Job drawing, mm, ordinate dimensions from the low corner. One solid piece. Give positions to 0.01 mm unless a question says otherwise; leave off trailing zeros. Loops run counter-clockwise (first coordinate to the right, second up) from the corner with the lowest first, then second, coordinate; pieces in that order, holes last.
Item 1: Saw through at B-B on x = 245. Give the cut face in (y, z).
Item 2: Probe probe 1 along Y at (x, z) = (245, 15); probe 2 along Y at (x, z) = (48, 21). List the from-to ranges inside material, lowest first.
Item 3: Drop a flat-ended pin along its axis: P1, Ø16, axis at x = 245, y = 110, coming from the +Z side. Give the stop position or say it passes through.
Item 4: Saw through at C-C on y = 30. Give the cut face in (x, z), plus the area to 3 significant figures.
Item 5: Saw through at A-A on z = 24.5. Give the cut face in (x, y), plus the area to 3 significant figures.
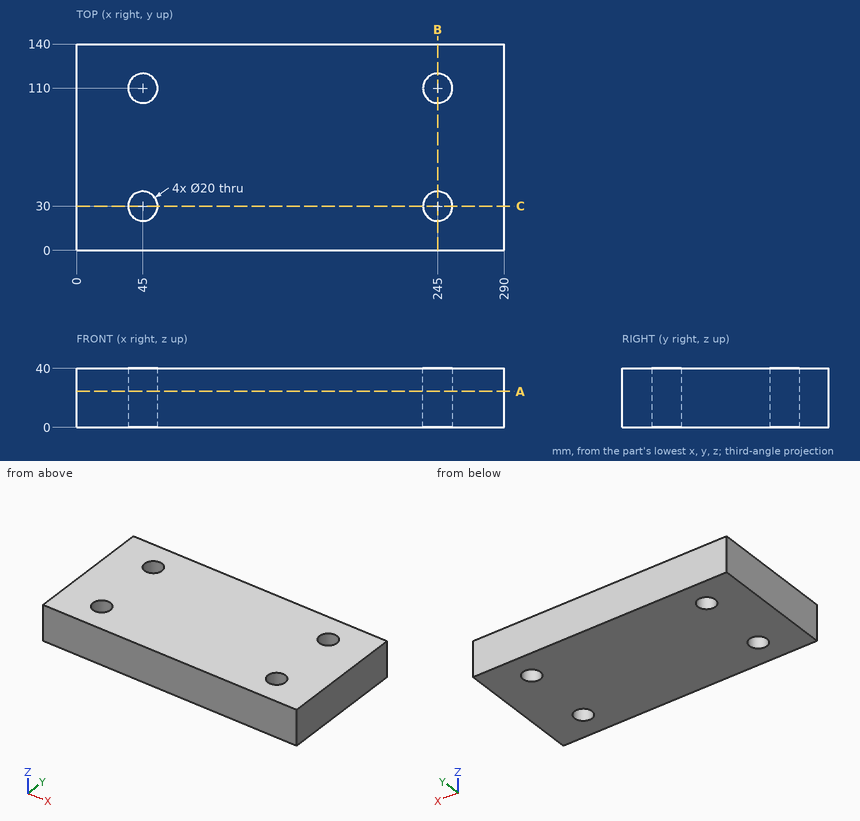
Results below:
1. outline: (0, 0) - (20, 0) - (20, 40) - (0, 40) - close; (40, 0) - (100, 0) - (100, 40) - (40, 40) - close; (120, 0) - (140, 0) - (140, 40) - (120, 40) - close
2. probe 1: y = 0 to 20, 40 to 100, 120 to 140
2. probe 2: y = 0 to 20.46, 39.54 to 100.46, 119.54 to 140
3. P1: passes through
4. outline: (0, 0) - (35, 0) - (35, 40) - (0, 40) - close; (55, 0) - (235, 0) - (235, 40) - (55, 40) - close; (255, 0) - (290, 0) - (290, 40) - (255, 40) - close
4. area: 10,000 mm2
5. outline: (0, 0) - (290, 0) - (290, 140) - (0, 140) - close; hole circle Ø20 at (45, 30); hole circle Ø20 at (45, 110); hole circle Ø20 at (245, 30); hole circle Ø20 at (245, 110)
5. area: 39,300 mm2
